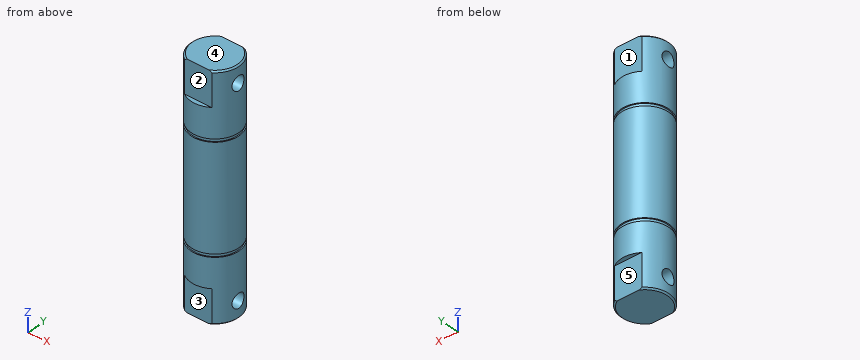
```python
from build123d import *

# Parameters (mm, degrees)
SKETCH_1_R          = 8.5
EXTRUDE_1_DEPTH     = 42
SKETCH_2_W          = 25
SKETCH_2_H          = 3
CUT_EXTRUDE_1_DEPTH = 12
CHAMFER_2_SIZE      = 0.5
HOLE_WIZARD_M6_1_D  = 5
SKETCH_5_W          = 0.4
SKETCH_5_H          = 1.1


with BuildPart() as part:
    # 草图1 → 凸台-拉伸1 (new, symmetric)
    with BuildSketch(Plane.XY):
        with Locations(Location((0, 0, 0), (0, 0, 180))):
            Circle(SKETCH_1_R)
    extrude(amount=EXTRUDE_1_DEPTH, both=True)

    # 草图2 → 切除-拉伸1 (cut)
    with BuildSketch(Plane.XY.offset(42)):
        with Locations((0, 8.5)):
            Rectangle(SKETCH_2_W, SKETCH_2_H)
        with Locations((0, -8.5)):
            Rectangle(SKETCH_2_W, SKETCH_2_H)
    cut_extrude_1 = extrude(amount=-CUT_EXTRUDE_1_DEPTH, mode=Mode.SUBTRACT)

    # 镜向1: 切除-拉伸1 across plane
    add(cut_extrude_1.mirror(Plane.XY), mode=Mode.SUBTRACT)

    # 倒角2
    chamfer_2_edges = [part.edges().sort_by_distance(p)[0] for p in [
        (8.5, 0, 42),
        (-7.524477249, 3.953763034, -42),
        (8.5, 0, -42),
        (-7.524477249, 3.953763034, 42),
    ]]
    chamfer(chamfer_2_edges, length=CHAMFER_2_SIZE)

    # M6 螺纹孔1 (through all)
    with Locations(Plane(origin=(8.5, 0, 0), x_dir=(0, 0, -1), z_dir=(1, 0, 0))):
        with Locations((-36, 0), (36, 0)):
            Hole(HOLE_WIZARD_M6_1_D / 2)

    # 草图5 → 切除-旋转1 (revolve, cut)
    with BuildSketch(Plane(origin=(0, 0, 0), x_dir=(1, 0, 0), z_dir=(0, 1, 0)), mode=Mode.PRIVATE) as cut_revolve_1_sk:
        with Locations((-8.3, 19.05)):
            Rectangle(SKETCH_5_W, SKETCH_5_H)
        with Locations((-8.3, -19.05)):
            Rectangle(SKETCH_5_W, SKETCH_5_H)
    revolve(cut_revolve_1_sk.sketch.rotate(Axis((0, 0, 0), (0, 0, -1)), 180), axis=Axis((0, 0, 0), (0, 0, -1)), mode=Mode.SUBTRACT)


solid = part.part
```
The listing builds one solid part. Answer for the finished solid, in the listing's coordinates (mm). Face numbers are marked on the shaded views. A direction names the side the tool comes from. Coordinates: 2 decimals unless noted, no trailing zeros. Loops run counter-clockwise (first coordinate to the right, second up) from the corner with the lowest first, then second, coordinate; pieces in that order, holes last. Notation, with made-up numbers: M -5,36.25 L 48,36.25 A21 cw 48,53.25 Z; hole C 64.5,54 d6. An arc over 180 degrees is marked long. Answer as a JSON object with one key per item and string values. Group by question number.
Item 1: Each of these flat-tipped pins is pushed along its axis until it touches: P1, Ø8, axis at y = 0, z = -36, coming from the -X side; P2, Ø2, axis at x = -5.5, z = -9.5, coming from the +Y side; P3, Ø1.6, axis at x = 2, y = -8, coming from the +Z side; P4, Ø0.8, axis at x = -2, y = -7.5, coming from the -Z side. Where does it stop, or does it pass through?
Item 2: Section C-C (z = 36) is taken. Write down the section's boundary in (x, y), and give its area (3 significant figures).
Item 3: Which of the six approach directions +Z, -Z, +X, -X, +Y, -Y give full straight-line access (tool end or side, diameter ignored) to the marked faces 1, 2, 3, 4 and 5?
Item 4: Section A-A (y = 0) is taken. Give the number of separate pieces and of enclosed holes in the cut face, and give its area (3 significant figures).
Item 5: Consider L1, parallel to Z at x = 3, y = 0; L2, parallel to Y at x = -0.5, z = -36; L3, parallel to X at y = -0.5, z = 12.5. Determine where each line is inside the solid, lowest interval first.
Item 6: Section D-D (z = -1) is taken. Write down the section's boundary in (x, y).
Solved:
{
 "1": {"P1": "stops at x = -8.5", "P2": "stops at y = 7.21", "P3": "stops at z = 30", "P4": "stops at z = -30"},
 "2": {"outline": "M -8.12,-2.5 A8.5 ccw -4.82,-7 L 4.82,-7 A8.5 ccw 8.12,-2.5 Z; M -8.12,2.5 L 8.12,2.5 A8.5 ccw 4.82,7 L -4.82,7 A8.5 ccw Z", "area": "124 mm2"},
 "3": {"face 1": "+Z, +X, -X, +Y", "face 2": "+Z, +X, -X, -Y", "face 3": "-Z, +X, -X, -Y", "face 4": "+Z, +X, -X, +Y, -Y", "face 5": "-Z, +X, -X, +Y"},
 "4": {"separate pieces": "3", "enclosed holes": "0", "area": "1,260 mm2"},
 "5": {"L1": "z = -42 to -38.5, -33.5 to 33.5, 38.5 to 42", "L2": "y = -7 to -2.5, 2.5 to 7", "L3": "x = -8.49 to 8.49"},
 "6": {"outline": "C 0,0 d17"}
}
